For this review, take the finished solid that the model builds, in its own axes (mm). Face numbers are marked on the shaded views. A direction names the side the tool comes from. Give positions to 0.01 mm unless a question says otherwise; leave off trailing zeros. Order: outer loops, then holes, each group sorted by start corner. A loop starts at its lowest first (then second) coordinate and runs counter-clockwise, first axis right, second up.
Item 1: Consider section A-A (z = -13.5). Give the boundary of the cut face in (x, y).
Item 2: Machinability: for the marked faces 1 and 2, which of the approach directions +Z, -Z, +X, -X, +Y, -Y give a long, thin tool a straight path to every point of the face, cutting with its end or side? Answer none if there is none.
Item 3: For probe 1 along Z at (x, y) = (0, 9.25); probe 2 along X at (y, z) = (108, -13.5); probe 3 along Y at (x, z) = (-4, -15.5), list the stretches that pass through material, from the lowest coordinate up.
Item 4: Consider section B-B (y = 53). Give the boundary of the cut face in (x, z).
Item 5: For P1, Ø1.5, axis at x = 1.5, y = 76.5, coming from the -Z side; P2, Ø3, axis at x = 0, z = 3.5, coming from the -Y side, all flat-tipped, find the tip position at first contact; note any pin that passes through.
```python
from build123d import *

# Parameters (mm, degrees)
SKETCH1_W                   = 10
SKETCH1_H                   = 15
BOSS_EXTRUDE1_DEPTH         = 114
SKETCH2_W                   = 10
SKETCH2_H                   = 10
SKETCH2_R                   = 3.1
BOSS_EXTRUDE2_DEPTH         = 10
M4_TAPPED_HOLE1_D           = 3.3
M4_TAPPED_HOLE1_DEPTH       = 11.5
M4_TAPPED_HOLE1_CSINK_D     = 4.05
M4_TAPPED_HOLE1_CSINK_ANGLE = 90
M4_TAPPED_HOLE1_TIP         = 0.991420021


with BuildPart() as part:
    # Sketch1 → Boss-Extrude1 (new body)
    with BuildSketch(Plane(origin=(0, 0, 0), x_dir=(1, 0, 0), z_dir=(0, 1, 0))):
        Rectangle(SKETCH1_W, SKETCH1_H)
    extrude(amount=BOSS_EXTRUDE1_DEPTH)

    # Sketch2 → Boss-Extrude2 (add)
    with BuildSketch(Plane(origin=(0, 114, 0), x_dir=(1, 0, 0), z_dir=(0, 1, 0))):
        with Locations((0, 12.5)):
            Rectangle(SKETCH2_W, SKETCH2_H)
        with Locations(Location((0, 13.5, 0), (0, 0, 270))):
            Circle(SKETCH2_R, mode=Mode.SUBTRACT)
    extrude(amount=-BOSS_EXTRUDE2_DEPTH)

    # M4 Tapped Hole1
    with Locations(Plane(origin=(0, 0, 0), x_dir=(-1, 0, 0), z_dir=(0, -1, 0))):
        with Locations((0, 3.5), (0, -3.5)):
            CounterSinkHole(M4_TAPPED_HOLE1_D / 2, M4_TAPPED_HOLE1_CSINK_D / 2, depth=M4_TAPPED_HOLE1_DEPTH, counter_sink_angle=M4_TAPPED_HOLE1_CSINK_ANGLE)
            with Locations((0, 0, -(M4_TAPPED_HOLE1_DEPTH + M4_TAPPED_HOLE1_TIP / 2))):  # 118° drill point
                Cone(0, M4_TAPPED_HOLE1_D / 2, M4_TAPPED_HOLE1_TIP, mode=Mode.SUBTRACT)


solid = part.part
```
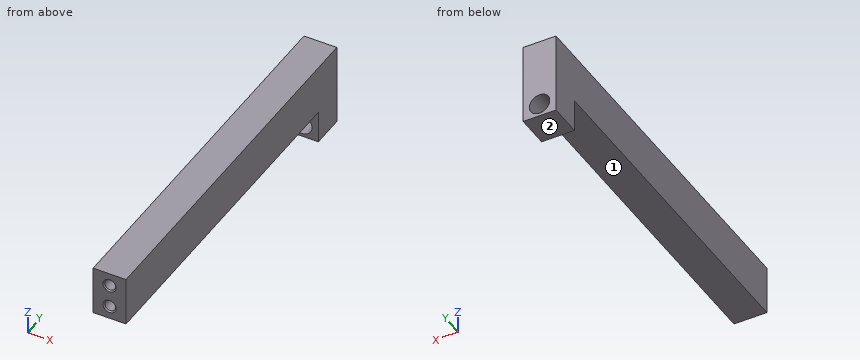
Resolved:
1. outline: (-5, 104) - (-3.1, 104) - (-3.1, 114) - (-5, 114) - close; (3.1, 104) - (5, 104) - (5, 114) - (3.1, 114) - close
2. face 1: -Z, +X, -X, -Y
2. face 2: -Z, +X, -X, +Y, -Y
3. probe 1: z = -7.5 to -5.15, -1.85 to 1.85, 5.15 to 7.5
3. probe 2: x = -5 to -3.1, 3.1 to 5
3. probe 3: y = 104 to 114
4. outline: (-5, -7.5) - (5, -7.5) - (5, 7.5) - (-5, 7.5) - close
5. P1: stops at z = -7.5
5. P2: stops at y = 11.59
